Drawing for the job (mm, zero at the part's lowest x, y, z). A direction names the side the tool comes from. Give positions to 0.01 mm unless a question says otherwise; leave off trailing zeros. Order: outer loops, then holes, each group sorted by start corner. A loop starts at its lowest first (then second) coordinate and runs counter-clockwise, first axis right, second up. Notation, with made-up numbers: M 82.5,10 L 121.5,10 A22 ccw 121.5,37 Z; hole C -4.75,21.25 d6. An arc over 180 degrees is marked long. Answer as a JSON object with one key per item and string values.
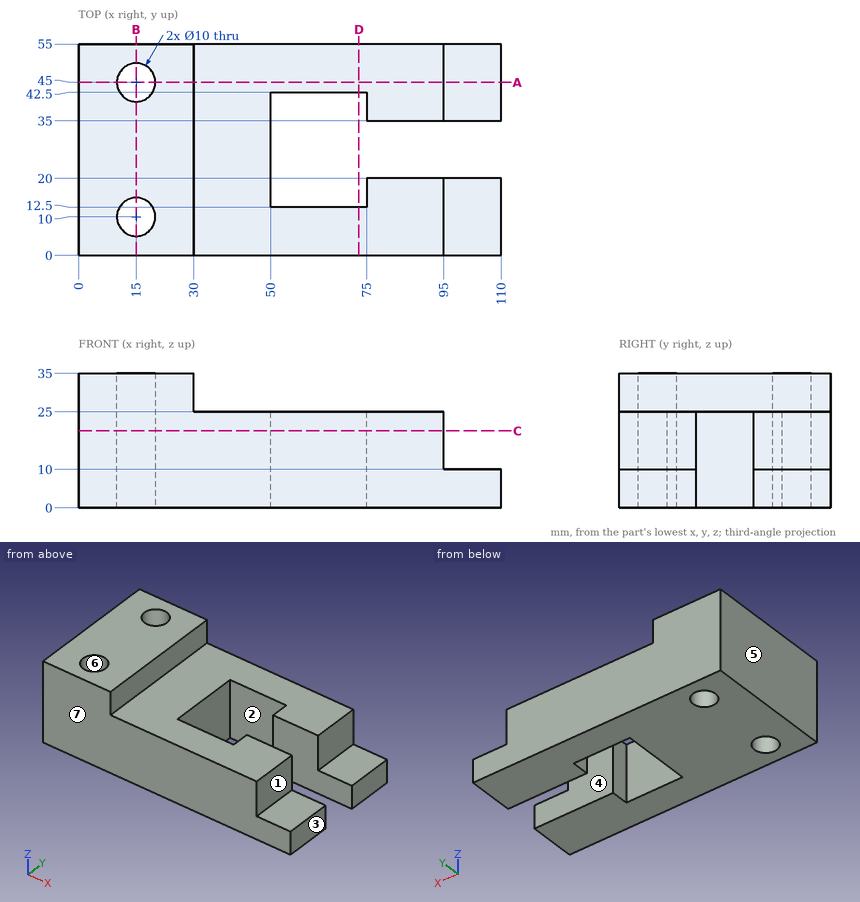
1. Cut at B-B on x = 15. Give the cut face in (y, z).
Worked answers:
{"outline": "M 0,0 L 5,0 L 5,35 L 0,35 Z; M 15,0 L 40,0 L 40,35 L 15,35 Z; M 50,0 L 55,0 L 55,35 L 50,35 Z"}
2. Probe line 1 along Y through (x, z) = (15, 17); line 2 along Y through (x, z) = (50.5, 10); line 3 along Z through (x, y) = (89, 4.5). List the from-to ranges inside material, lowest first.
Worked answers:
{"line 1": "y = 0 to 5, 15 to 40, 50 to 55", "line 2": "y = 0 to 12.5, 42.5 to 55", "line 3": "z = 0 to 25"}
3. Cut at C-C on z = 20. Give the cut face in (x, y), plus the area to 3 significant figures.
Worked answers:
{"outline": "M 0,0 L 95,0 L 95,20 L 75,20 L 75,12.5 L 50,12.5 L 50,42.5 L 75,42.5 L 75,35 L 95,35 L 95,55 L 0,55 Z; hole C 15,10 d10; hole C 15,45 d10", "area": "4,020 mm^2"}
4. Two-plate mould, pull along Y, no slides. Class the marked faces 5, 6 and 7: +Y half, -Y half, draft (parallel to the pull), parting line (faces both ways), or undercut.
Worked answers:
{"face 5": "draft", "face 6": "undercut", "face 7": "-Y half"}
5. Which spindle directions (+Z, -Z, +X, -X, +Y, -Y) get a long thin tool onto all of the face, cutting with end or side? Do the marked faces 1, 2, 3 and 4. Say none if no direction does.
Worked answers:
{"face 1": "+Z, +X, +Y, -Y", "face 2": "+Z, -Z", "face 3": "+Z, -Z, +X, +Y, -Y", "face 4": "+Z, -Z, +X"}
6. Cut at D-D on x = 73. Give the cut face in (y, z).
Worked answers:
{"outline": "M 0,0 L 12.5,0 L 12.5,25 L 0,25 Z; M 42.5,0 L 55,0 L 55,25 L 42.5,25 Z"}
7. Pin check, flat tips, straight feed: P1, Ø1, axis at x = 33.5, y = 43.5, coming from the -Z side; P2, Ø16.5, axis at x = 71, y = 21, coming from the +Z side; P3, Ø12, axis at x = 104, y = 43.5, coming from the +Z side; P4, Ø5, axis at y = 16.5, z = 30, coming from the +X side. Stop position of each tip, or through.
Worked answers:
{"P1": "stops at z = 0", "P2": "stops at z = 25", "P3": "stops at z = 10", "P4": "stops at x = 30"}
8. Cut at A-A on y = 45. Give the cut face in (x, z).
Worked answers:
{"outline": "M 0,0 L 10,0 L 10,35 L 0,35 Z; M 20,0 L 110,0 L 110,10 L 95,10 L 95,25 L 30,25 L 30,35 L 20,35 Z"}
